Design review of the part shown in the three views and the two pictorial views. Dimensions are in mm from the part's minimum x, y and z. A direction names the side the tool comes from. Round coordinates to 2 decimals unless told otherwise and drop trailing zeros. Order: outer loops, then holes, each group sorted by start corner. A loop starts at its lowest first (then second) coordinate and runs counter-clockwise, first axis right, second up.
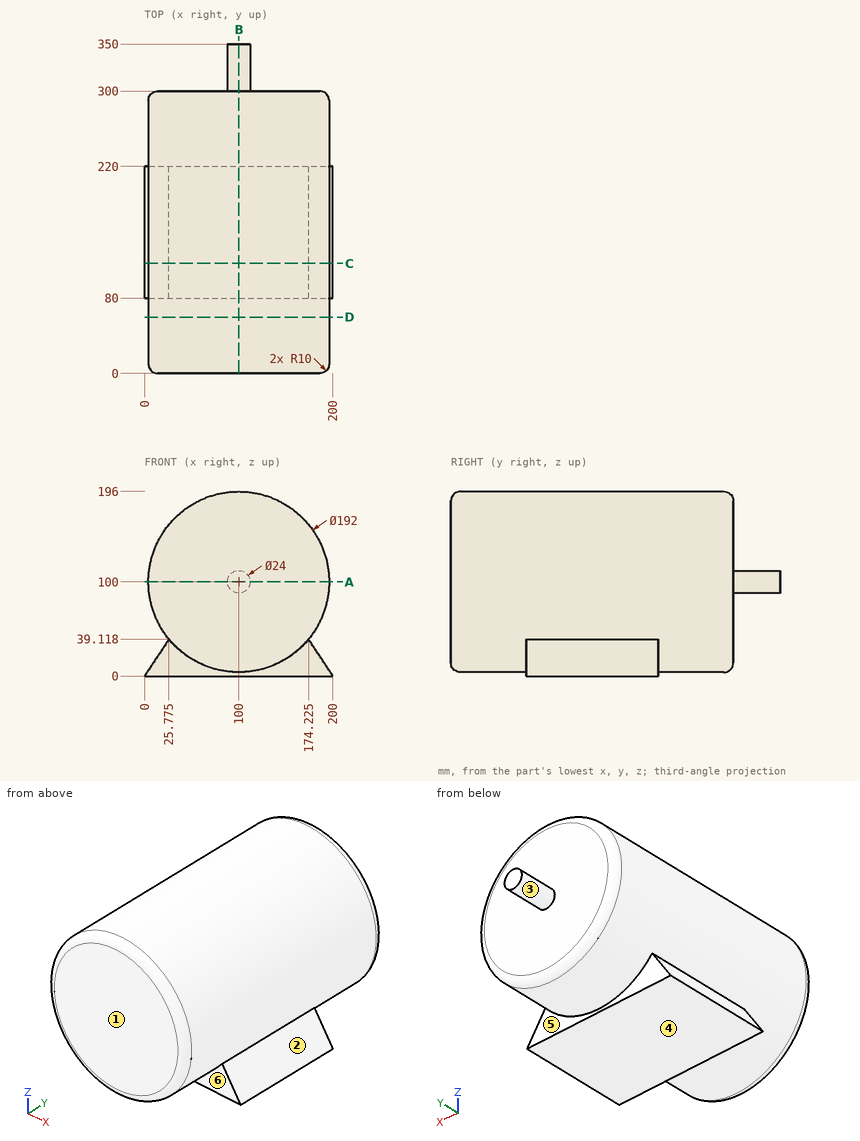
(1) Add section D-D on y = 60. Give the boundary of the cut face in (x, z), plus the area to 3 significant figures.
(2) Add section B-B on x = 100. Give the boundary of the cut face in (y, z), plus the area to 3 significant figures.
(3) Draft analysis for pull direction Z (two halves, no side actions). For the marked faces 1, 2 and 3, state which applies: pulls with the +Z half, pulls with the -Z half, needs draft (parallel to the pull), parting line crosses it, or undercut.
(4) Wall thickness on L1, parallel to X at y = 68.5, z = 99.5; L2, parallel to Y at x = 106, z = 151.5; L3, parallel to Z at x = 181, y = 124.5 (1 decimal): over which ranges is each line inside the solid? List them lowest first.
(5) Clearance check with flat-ended pins moving along their axes: P1, Ø8, axis at x = 47.5, z = 52, coming from the +Y side; P2, Ø1.5, axis at y = 140, z = 48.5, coming from the -X side; P3, Ø1, axis at y = 198.5, z = 155, coming from the -X side. State where each tip first meets the part, or that it passes through.
(6) Tool access review of the marked faces 4, 5 and 6: name each direction out of +Z, -Z, +X, -X, +Y, -Y from which nothing blocks a thin tool from reaching the whole face with its end or side.
(7) Add section A-A on z = 100. Give the boundary of the cut face in (x, y), plus the area to 3 significant figures.
(8) Add section C-C on y = 117. Give the boundary of the cut face in (x, z) (1 decimal).
Here are the results:
1. outline: circle Ø192 at (100, 100)
1. area: 29,000 mm2
2. outline: (0, 14) arc R10 ccw to (10, 4) - (80, 4) - (80, 0) - (220, 0) - (220, 4) - (290, 4) arc R10 ccw to (300, 14) - (300, 88) - (350, 88) - (350, 112) - (300, 112) - (300, 186) arc R10 ccw to (290, 196) - (10, 196) arc R10 ccw to (0, 186) - close
2. area: 59,300 mm2
3. face 1: needs draft
3. face 2: undercut
3. face 3: parting line crosses it
4. L1: x = 4 to 196
4. L2: y = 0 to 300
4. L3: z = 0 to 28.8, 48.5 to 151.5
5. P1: stops at y = 300
5. P2: stops at x = 18.51
5. P3: stops at x = 20.97
6. face 4: -Z, +X, -X, +Y, -Y
6. face 5: -Z, +Y
6. face 6: -Z, -Y
7. outline: (4, 10) arc R10 ccw to (14, 0) - (186, 0) arc R10 ccw to (196, 10) - (196, 290) arc R10 ccw to (186, 300) - (112, 300) - (112, 350) - (88, 350) - (88, 300) - (14, 300) arc R10 ccw to (4, 290) - close
7. area: 58,700 mm2
8. outline: (0, 0) - (200, 0) - (174.2, 39.1) arc R96 ccw (long way) to (25.8, 39.1) - close
